Work out the finished part from the listing and answer in its coordinate system (mm). Face numbers are marked on the shaded views. A direction names the side the tool comes from. Coordinates: 2 decimals unless noted, no trailing zeros. Write each loop counter-clockwise with the first axis right and the second up, starting at its lowest first coordinate (ties: lowest second). Pieces come first, ordered by that corner, then holes. Notation, with made-up numbers: M -32,81.25 L -9,81.25 A11 cw -9,94.25 Z; hole C 75.5,31 d2. An arc over 180 degrees is marked long. Answer as CSV lines item,"result". Start each with the question number.
(1) Flat-ended cylindrical pins translate along their axes: P1, Ø1.5, axis at x = 16.5, y = 18, coming from the -Z side; P2, Ø13, axis at x = 33.5, y = 40, coming from the -Z side; P3, Ø1.5, axis at y = 35, z = -24, coming from the +X side. Find the tip coordinate at first contact, or state that the pin passes through.
(2) A cutting plane is placed at B-B on z = -24. Give the vertices of the cut face in (x, y), then the cut area to 3 significant figures.
(3) A cutting plane is placed at A-A on y = 22. Give the vertices of the cut face in (x, z).
(4) A cutting plane is placed at D-D on y = 36.5. Give the vertices of the cut face in (x, z).
(5) Find the intervals of material crossed by L1, parallel to Z at x = 40, y = 9.25; L2, parallel to X at y = 39, z = -24; L3, parallel to Y at x = 32.5, z = -46, in increasing order. Write a range as [from, to].
(6) The mould has two halves that part along Y. Classify the marked faces 1, 2 and 3: released by +Y, released by -Y, zero draft, split by the parting line, or undercut.
(7) A cutting plane is placed at C-C on x = 52. Give the vertices of the cut face in (y, z), then the cut area to 3 significant figures.
(8) For the marked faces 4, 5, 6 and 7, determine the directions among +Z, -Z, +X, -X, +Y, -Y from which every point of the face is accessible in a straight line to the end or side of a thin tool.
from build123d import *

# Parameters (mm, degrees)
BASE_BLOCK_DEPTH             = 16
BASE_WINDOW_CUT_DEPTH        = 16
FIRST_LUG_DEPTH              = 12
SECOND_START                 = -12
SECOND_LUG_DEPTH             = 12
SECOND_LUG_HOLE_PROFILE_20_R = 10
SECOND_LUG_PIN_HOLE_20_DEPTH = 12
FIRST_START                  = -12
FIRST_LUG_HOLE_PROFILE_20_R  = 10
FIRST_LUG_PIN_HOLE_20_DEPTH  = 12
FIRST_LUG_FILLETS_R2_R       = 2
LUG_JUNCTION_FILLETS_R2_R    = 2
WINDOW_EDGE_FILLETS_R2_R     = 2


with BuildPart() as part:
    # Base Block Profile → Base Block (new body)
    with BuildSketch(Plane(origin=(0, 0, 0), x_dir=(0, 0, -1), z_dir=(1, 0, 0))):
        with BuildLine():
            Line((0, 0), (0, 44))
            Line((0, 44), (96, 44))
            ThreePointArc((96, 44), (118, 22), (96, 0))
            Line((96, 0), (0, 0))
        make_face()
    extrude(amount=BASE_BLOCK_DEPTH)

    # Window Profile → Base Window Cut (cut)
    with BuildSketch(Plane(origin=(16, 0, 0), x_dir=(0, 0, -1), z_dir=(1, 0, 0))):
        with BuildLine():
            Line((72, 30), (96, 30))
            ThreePointArc((96, 30), (104, 22), (96, 14))
            Line((96, 14), (72, 14))
            ThreePointArc((72, 14), (64, 22), (72, 30))
        make_face()
    extrude(amount=-BASE_WINDOW_CUT_DEPTH, mode=Mode.SUBTRACT)

    # First Lug Profile → First Lug (add)
    with BuildSketch(Plane.XZ):
        with BuildLine():
            Line((0, 0), (40, 0))
            ThreePointArc((40, 0), (64, -24), (40, -48))
            Line((40, -48), (0, -48))
            Line((0, -48), (0, 0))
        make_face()
    extrude(amount=-FIRST_LUG_DEPTH)

    # Second Lug Profile → Second Lug (add)
    with BuildSketch(Plane(origin=(0, 44, 0), x_dir=(1, 0, 0), z_dir=(0, 1, 0)).offset(SECOND_START)):
        with BuildLine():
            Line((0, 0), (40, 0))
            ThreePointArc((40, 0), (64, 24), (40, 48))
            Line((40, 48), (0, 48))
            Line((0, 48), (0, 0))
        make_face()
    extrude(amount=SECOND_LUG_DEPTH)

    # Second Lug Hole Profile Ø20 → Second Lug Pin Hole Ø20 (cut)
    with BuildSketch(Plane(origin=(0, 44, 0), x_dir=(1, 0, 0), z_dir=(0, 1, 0))):
        with Locations(Location((40, 24, 0), (0, 0, 270))):
            Circle(SECOND_LUG_HOLE_PROFILE_20_R)
    extrude(amount=-SECOND_LUG_PIN_HOLE_20_DEPTH, mode=Mode.SUBTRACT)

    # First Lug Hole Profile Ø20 → First Lug Pin Hole Ø20 (cut)
    with BuildSketch(Plane.XZ.offset(FIRST_START)):
        with Locations(Location((40, -24, 0), (0, 0, 90))):
            Circle(FIRST_LUG_HOLE_PROFILE_20_R)
    extrude(amount=FIRST_LUG_PIN_HOLE_20_DEPTH, mode=Mode.SUBTRACT)

    # First Lug Fillets R2
    first_lug_fillets_r2_edges = [part.edges().sort_by_distance(p)[0] for p in [
        (16, 6, -48),
    ]]
    fillet(first_lug_fillets_r2_edges, radius=FIRST_LUG_FILLETS_R2_R)

    # Lug Junction Fillets R2
    lug_junction_fillets_r2_edges = [part.edges().sort_by_distance(p)[0] for p in [
        (16, 12, -25),
        (16, 32, -24),
        (16, 38, -48),
    ]]
    fillet(lug_junction_fillets_r2_edges, radius=LUG_JUNCTION_FILLETS_R2_R)

    # Window Edge Fillets R2
    window_edge_fillets_r2_edges = [part.edges().sort_by_distance(p)[0] for p in [
        (16, 22, -64),
        (16, 14, -84),
        (16, 22, -104),
        (16, 30, -84),
    ]]
    fillet(window_edge_fillets_r2_edges, radius=WINDOW_EDGE_FILLETS_R2_R)


solid = part.part
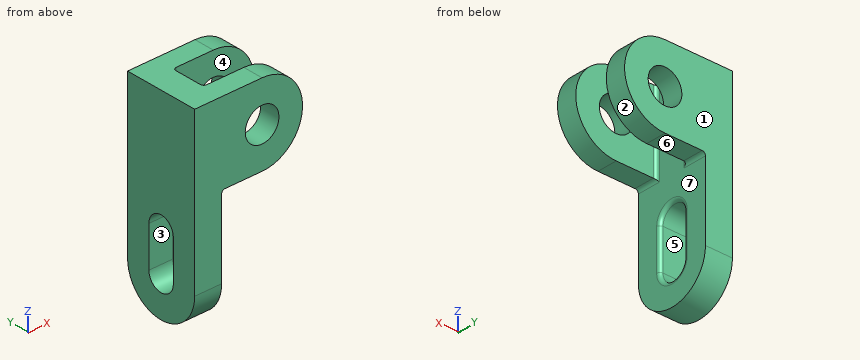
Here are the results:
1,P1,"stops at z = -117.73"
1,P2,"stops at z = -48"
1,P3,"stops at x = 64"
2,outline,"M 0,0 L 30,0 L 30,12 L 18,12 A2 cw 16,14 L 16,30 A2 cw 18,32 L 30,32 L 30,44 L 0,44 Z; M 50,0 L 64,0 L 64,12 L 50,12 Z; M 50,32 L 64,32 L 64,44 L 50,44 Z"
2,area,"1,380 mm^2"
3,outline,"M 0,-118 L 16,-118 L 16,-106 A2 ccw 14,-104 L 0,-104 Z; M 0,-64 L 14,-64 A2 ccw 16,-62 L 16,0 L 0,0 Z"
4,outline,"M 0,-112.55 L 16,-112.55 L 16,-50 A2 cw 18,-48 L 40,-48 A24 ccw 40,0 L 0,0 Z; hole C 40,-24 d20"
5,L1,"z = [-48, -34], [-14, 0]"
5,L2,"x = [0, 30], [50, 64]"
5,L3,"y = [0, 12], [32, 44]"
6,face 1,"released by +Y"
6,face 2,"zero draft"
6,face 3,"undercut"
7,outline,"M 0,-44.78 L 12,-44.78 L 12,-3.22 L 0,-3.22 Z; M 32,-44.78 L 44,-44.78 L 44,-3.22 L 32,-3.22 Z"
7,area,"998 mm^2"
8,face 4,"+Z, -Z, +X"
8,face 5,"+X, -X"
8,face 6,"-Z, +X, +Y, -Y"
8,face 7,"-Z, +X"
